Input: part model. Units: mm. Frame: model coordinates. Face numbers are marked on the shaded views. Coordinates: 2 decimals unless noted, no trailing zeros. Loops run counter-clockwise (first coordinate to the right, second up) from the corner with the lowest first, then second, coordinate; pieces in that order, holes last. Notation, with made-up numbers: (1.25, 65.5) -> (35.25, 65.5) arc R22 ccw to (35.25, 78.5) -> close; hole circle Ø4 at (62.5, -23.5). An arc over 180 degrees is marked (long way). Put each result on its own line as item: value. Start each with the question number.
1) Contact query for flat-ended pins moving along their axis: P1, Ø5.5, axis at x = -43.5, y = -9.5, coming from the +Z side; P2, Ø14.5, axis at x = -0.74, y = -8.85, coming from the -Z side; P3, Ø12, axis at x = 1, y = -6, coming from the +Z side. Output: stop coordinate, or through.
2) Cut plane D-D (z = 10). Return the cut outline in (x, y), plus the area to 3 significant figures.
3) Pull-direction query (Z, two-part tool) for the marked faces 1, 2 and 3; classes: pulls with the +Z half, pulls with the -Z half, needs draft (parallel to the pull), parting line crosses it, or undercut.
4) Cut plane B-B (y = -10.5). Return the cut outline in (x, z).
5) Cut plane A-A (x = -22). Return the cut outline in (y, z).
6) Cut plane C-C (z = 25). Return the cut outline in (x, y), plus the area to 3 significant figures.
7) Material intervals for L1, parallel to Y at x = -51, z = 35; L2, parallel to Y at x = -9, z = 29; L3, parallel to Z at x = 1.5, y = 5.5, sorted ascending.
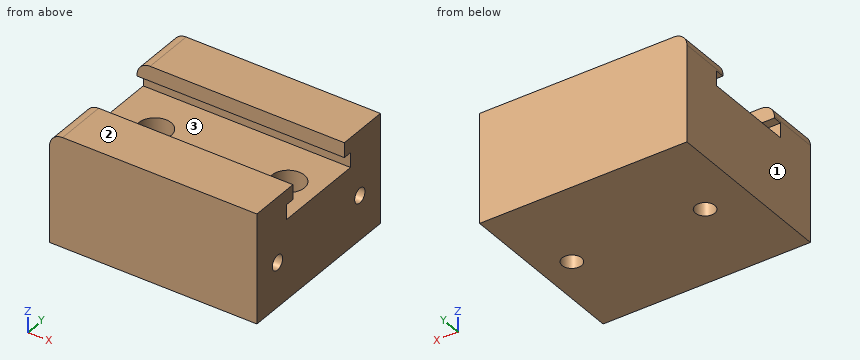
from build123d import *

# Parameters (mm, degrees)
SKETCH1_W                                           = 70
SKETCH1_H                                           = 60
BOSS_EXTRUDE1_DEPTH                                 = 37
CUT_EXTRUDE2_DEPTH                                  = 89.196341816
M6_TAPPED_HOLE1_D                                   = 5
M6_TAPPED_HOLE1_DEPTH                               = 15
M6_TAPPED_HOLE1_TIP                                 = 1.502151548
FILLET1_R                                           = 4.4
CBORE_FOR_M6_HEX_SOCKET_HEAD_CAP_SCREW1_D           = 6.6
CBORE_FOR_M6_HEX_SOCKET_HEAD_CAP_SCREW1_CBORE_D     = 11
CBORE_FOR_M6_HEX_SOCKET_HEAD_CAP_SCREW1_CBORE_DEPTH = 25


with BuildPart() as part:
    # Sketch1 → Boss-Extrude1 (new body)
    with BuildSketch(Plane.XY):
        with Locations((-25.437479048, -8.853503185)):
            Rectangle(SKETCH1_W, SKETCH1_H)
    extrude(amount=BOSS_EXTRUDE1_DEPTH)

    # Sketch3 → Cut-Extrude2 (cut, through all)
    with BuildSketch(Plane(origin=(9.562520952, 0, 0), x_dir=(0, 0, -1), z_dir=(1, 0, 0))):
        Polygon((-32, -24.353503185), (-27, -24.353503185), (-27, 6.646496815), (-32, 6.646496815), (-32, 3.646496815), (-37, 3.646496815), (-37, -21.353503185), (-32, -21.353503185), align=None)
    extrude(amount=-CUT_EXTRUDE2_DEPTH, mode=Mode.SUBTRACT)

    # M6 Tapped Hole1
    with Locations(Plane(origin=(9.562520952, 0, 0), x_dir=(0, 0, -1), z_dir=(1, 0, 0))):
        with Locations((-15, -28.853503185), (-15, 11.146496815)):
            Hole(M6_TAPPED_HOLE1_D / 2, depth=M6_TAPPED_HOLE1_DEPTH)
            with Locations((0, 0, -(M6_TAPPED_HOLE1_DEPTH + M6_TAPPED_HOLE1_TIP / 2))):  # 118° drill point
                Cone(0, M6_TAPPED_HOLE1_D / 2, M6_TAPPED_HOLE1_TIP, mode=Mode.SUBTRACT)

    # Fillet1
    fillet1_edges = [part.edges().sort_by_distance(p)[0] for p in [
        (-60.437479048, -30.103503185, 37),
        (-60.437479048, 12.396496815, 37),
    ]]
    fillet(fillet1_edges, radius=FILLET1_R)

    # CBORE for M6 Hex Socket Head Cap Screw1 (through all)
    with Locations(Plane.XY.offset(37)):
        with Locations((-0.737479048, -8.853503185), (-45.737479048, -8.853503185)):
            CounterBoreHole(CBORE_FOR_M6_HEX_SOCKET_HEAD_CAP_SCREW1_D / 2, CBORE_FOR_M6_HEX_SOCKET_HEAD_CAP_SCREW1_CBORE_D / 2, CBORE_FOR_M6_HEX_SOCKET_HEAD_CAP_SCREW1_CBORE_DEPTH)


solid = part.part
Results found:
1. P1: stops at z = 12
1. P2: stops at z = 0
1. P3: stops at z = 27
2. outline: (-60.44, -38.85) -> (9.56, -38.85) -> (9.56, 21.15) -> (-60.44, 21.15) -> close; hole circle Ø6.6 at (-45.74, -8.85); hole circle Ø6.6 at (-0.74, -8.85)
2. area: 4,130 mm2
3. face 1: needs draft
3. face 2: pulls with the +Z half
3. face 3: undercut
4. outline: (-60.44, 0) -> (-48.6, 0) -> (-48.6, 12) -> (-50.99, 12) -> (-50.99, 27) -> (-60.44, 27) -> close; (-42.88, 0) -> (-3.6, 0) -> (-3.6, 12) -> (-5.99, 12) -> (-5.99, 27) -> (-40.49, 27) -> (-40.49, 12) -> (-42.88, 12) -> close; (2.12, 0) -> (9.56, 0) -> (9.56, 27) -> (4.51, 27) -> (4.51, 12) -> (2.12, 12) -> close
5. outline: (-38.85, 0) -> (21.15, 0) -> (21.15, 37) -> (3.65, 37) -> (3.65, 32) -> (6.65, 32) -> (6.65, 27) -> (-24.35, 27) -> (-24.35, 32) -> (-21.35, 32) -> (-21.35, 37) -> (-38.85, 37) -> close
6. outline: (-60.44, -38.85) -> (9.56, -38.85) -> (9.56, 21.15) -> (-60.44, 21.15) -> close; hole circle Ø11 at (-45.74, -8.85); hole circle Ø11 at (-0.74, -8.85)
6. area: 4,010 mm2
7. L1: y = -38.85 to -21.35, 3.65 to 21.15
7. L2: y = -38.85 to -24.35, 6.65 to 21.15
7. L3: z = 0 to 27, 32 to 37
